Geometry: see drawing. Coordinates: mm, zero at the bounding-box minimum. Round coordinates to 2 decimals unless told otherwise and drop trailing zeros. Loops run counter-clockwise (first coordinate to the right, second up) from the corner with the lowest first, then second, coordinate; pieces in that order, holes last. Notation, with made-up numbers: (58, 52) -> (97, 52) arc R31 ccw to (97, 77) -> close; hole circle Ø7 at (16, -22). An arc over 180 degrees is marked (long way). Answer in a Markdown table with one row per item.
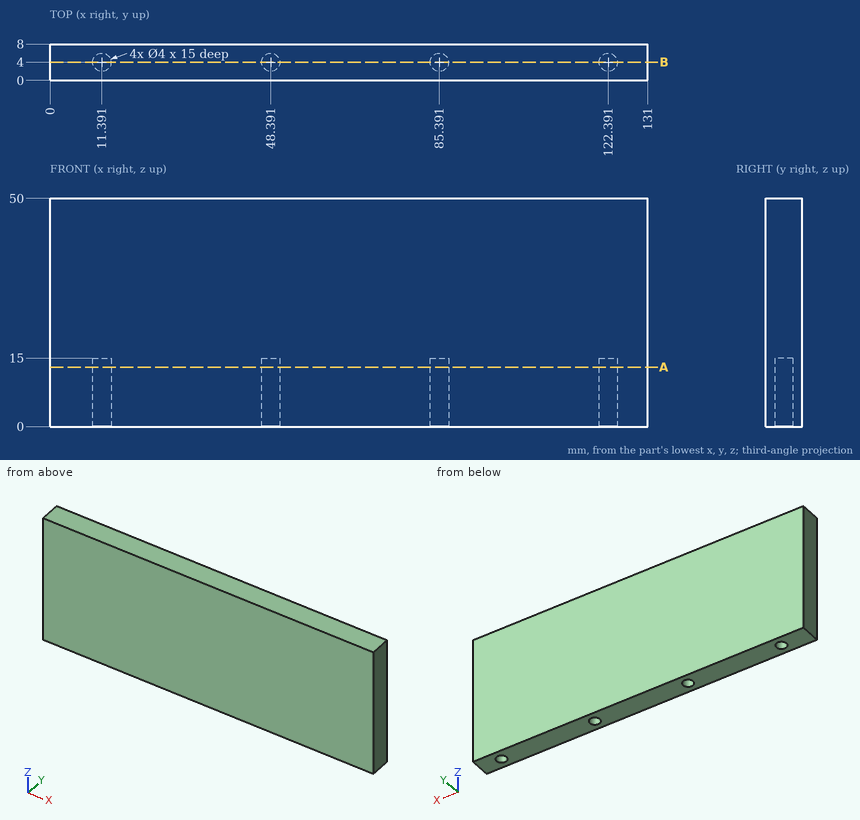
Item 1: Section query A-A, the plane z = 13. Output: boundary loops of the cut face in (x, y).
Ans:
| item | result |
|---|---|
| outline | (0, 0) -> (131, 0) -> (131, 8) -> (0, 8) -> close; hole circle Ø4 at (11.39, 4); hole circle Ø4 at (48.39, 4); hole circle Ø4 at (85.39, 4); hole circle Ø4 at (122.39, 4) |
Item 2: Section query B-B, the plane y = 4. Output: boundary loops of the cut face in (x, z), and give its area (3 significant figures).
Ans:
| item | result |
|---|---|
| outline | (0, 0) -> (9.39, 0) -> (9.39, 15) -> (13.39, 15) -> (13.39, 0) -> (46.39, 0) -> (46.39, 15) -> (50.39, 15) -> (50.39, 0) -> (83.39, 0) -> (83.39, 15) -> (87.39, 15) -> (87.39, 0) -> (120.39, 0) -> (120.39, 15) -> (124.39, 15) -> (124.39, 0) -> (131, 0) -> (131, 50) -> (0, 50) -> close |
| area | 6,310 mm2 |
Item 3: First-contact query: P1, Ø1.2, axis at x = 47.5, y = 4, coming from the -Z side; P2, Ø5, axis at x = 62.5, z = 34.5, coming from the -Y side. Flat tips, straight axial feed; report the tip coordinate or a pass-through.
Ans:
| item | result |
|---|---|
| P1 | z = 15 |
| P2 | y = 0 |
Item 4: Ray query, L1, parallel to X at y = 3, z = 4.5. Return the intervals inside material, ascending.
Ans:
| item | result |
|---|---|
| L1 | 0 to 9.66, 13.12 to 46.66, 50.12 to 83.66, 87.12 to 120.66, 124.12 to 131 |
